Verification items for the finished model (mm, model axes). A direction names the side the tool comes from. Round coordinates to 2 decimals unless told otherwise and drop trailing zeros. Order: outer loops, then holes, each group sorted by start corner. A loop starts at its lowest first (then second) coordinate and runs counter-clockwise, first axis right, second up. Notation, with made-up numbers: (-34, -3) -> (-13, -3) arc R11 ccw to (-13, 4) -> close; hole circle Ø8 at (68.5, 62.5). An arc over 180 degrees is marked (long way). Write item = value, one per line. Start each with the question number.
from build123d import *

# Parameters (mm, degrees)
SKETCH1_W             = 15
SKETCH1_H             = 80
BOSS_EXTRUDE1_DEPTH   = 16
SKETCH2_W             = 12
SKETCH2_H             = 29.2
CUT_EXTRUDE1_DEPTH    = 46.617978912
M4_TAPPED_HOLE1_D     = 3.3
M4_TAPPED_HOLE1_DEPTH = 22.25
M4_TAPPED_HOLE1_TIP   = 0.991420021
CHAMFER1_SIZE         = 5
CHAMFER1_SIZE2        = 2.886751346
SKETCH6_R             = 15
CUT_EXTRUDE2_DEPTH    = 46.617978912


with BuildPart() as part:
    # Sketch1 → Boss-Extrude1 (new body)
    with BuildSketch(Plane.XY):
        Rectangle(SKETCH1_W, SKETCH1_H)
    extrude(amount=BOSS_EXTRUDE1_DEPTH)

    # Sketch2 → Cut-Extrude1 (cut, through all)
    with BuildSketch(Plane(origin=(7.5, 0, 0), x_dir=(0, 0, -1), z_dir=(1, 0, 0))):
        with Locations((-6, -25.4)):
            Rectangle(SKETCH2_W, SKETCH2_H)
    extrude(amount=-CUT_EXTRUDE1_DEPTH, mode=Mode.SUBTRACT)

    # M4 Tapped Hole1
    with Locations(Plane(origin=(0, 0, 12), x_dir=(-1, 0, 0), z_dir=(0, 0, -1))):
        with Locations((0, -17.8), (0, -31.8)):
            Hole(M4_TAPPED_HOLE1_D / 2, depth=M4_TAPPED_HOLE1_DEPTH)
            with Locations((0, 0, -(M4_TAPPED_HOLE1_DEPTH + M4_TAPPED_HOLE1_TIP / 2))):  # 118° drill point
                Cone(0, M4_TAPPED_HOLE1_D / 2, M4_TAPPED_HOLE1_TIP, mode=Mode.SUBTRACT)

    # Chamfer1
    chamfer1_edges = [part.edges().sort_by_distance(p)[0] for p in [
        (0, 40, 0),
    ]]
    chamfer1_side = [part.faces().sort_by_distance(p)[0] for p in [
        (0, 14.6, 0),
    ]]
    chamfer(chamfer1_edges, length=CHAMFER1_SIZE, length2=CHAMFER1_SIZE2, reference=chamfer1_side[0])

    # Sketch6 → Cut-Extrude2 (cut, through all)
    with BuildSketch(Plane(origin=(7.5, 0, 0), x_dir=(0, 0, -1), z_dir=(1, 0, 0))):
        with Locations((-21, 22)):
            Circle(SKETCH6_R)
    extrude(amount=-CUT_EXTRUDE2_DEPTH, mode=Mode.SUBTRACT)


solid = part.part
(1) Cross-section at A-A (x = 0). Enter the section's corners in (y, z).
(2) Cross-section at D-D (x = 4.25). Enter the section's corners in (y, z), and give its area (3 significant figures).
(3) Set-up check for faces 4 (the flat face through (0, -10.8, 6)), 5 (the flat face through (0, -16, 16)): record each of +Z, -Z, +X, -X, +Y, -Y from which the full face is reachable in a straight line by a thin tool's end or side.
(4) Scan lines: line 1 along X through (y, z) = (-18, 14.5); line 2 along Y through (x, z) = (0, 13.5); line 3 along Y through (x, z) = (-5.25, 4.75). Record each from-to range of solid material in increasing order. Write a range as from..to.
(5) Depth check by flat-ended pin: pin 1 (8 mm diameter, centred on x = 1, y = -18, fed in from -Z); pin 2 (4.5 mm diameter, centred on x = 0, y = -17.8, fed in from +Z); pin 3 (3 mm diameter, centred on x = -3, y = 24, fed in from +Z). Enter the tip coordinate at first touch or a pass-through.
(6) Cross-section at B-B (y = -17.8). Enter the section's corners in (x, z), and give its area (3 significant figures).
(7) Draft check along Y on faces 1 (the flat face through (0, 40, 9)), 2 (the flat face through (7.5, 8, 8)), 3 (the cylindrical face through (-0.4, -19.4, 14)). Enter one of: +Y half, -Y half, draft (parallel to the pull), parting line (faces both ways), or undercut.
(8) Cross-section at C-C (z = 13). Enter the section's corners in (x, y).
Outcome:
q1.outline = (-40, 12) -> (-33.45, 12) -> (-33.45, 16) -> (-40, 16) -> close; (-30.15, 12) -> (-19.45, 12) -> (-19.45, 16) -> (-30.15, 16) -> close; (-16.15, 12) -> (-10.8, 12) -> (-10.8, 0) -> (35, 0) -> (40, 2.89) -> (40, 16) -> (36.14, 16) arc R15 cw to (7.86, 16) -> (-16.15, 16) -> close
q2.outline = (-40, 12) -> (-10.8, 12) -> (-10.8, 0) -> (35, 0) -> (40, 2.89) -> (40, 16) -> (36.14, 16) arc R15 cw to (7.86, 16) -> (-40, 16) -> close
q2.area = 716 mm^2
q3.face_4 = -Z, +X, -X, -Y
q3.face_5 = +Z, +X, -X, +Y, -Y
q4.line_1 = -7.5..-1.64, 1.64..7.5
q4.line_2 = -40..-33.45, -30.15..-19.45, -16.15..9.01, 34.99..40
q4.line_3 = -10.8..40
q5.pin_1 = 12
q5.pin_2 = 16
q5.pin_3 = 6.41
q6.outline = (-7.5, 12) -> (-1.65, 12) -> (-1.65, 16) -> (-7.5, 16) -> close; (1.65, 12) -> (7.5, 12) -> (7.5, 16) -> (1.65, 16) -> close
q6.area = 46.8 mm^2
q7.face_1 = +Y half
q7.face_2 = draft
q7.face_3 = undercut
q8.outline = (-7.5, -40) -> (7.5, -40) -> (7.5, 9.31) -> (-7.5, 9.31) -> close; (-7.5, 34.69) -> (7.5, 34.69) -> (7.5, 40) -> (-7.5, 40) -> close; hole circle Ø3.3 at (0, -31.8); hole circle Ø3.3 at (0, -17.8)
